Build history of the part. All positions in model axes, mm. Face numbers are marked on the shaded views. A direction names the side the tool comes from. Give positions to 0.01 mm unless a question says otherwise; leave off trailing zeros. Loops run counter-clockwise (first coordinate to the right, second up) from the corner with the lowest first, then second, coordinate; pieces in that order, holes last. Notation, with made-up numbers: (59, -37) -> (92, -37) arc R11 ccw to (92, -32) -> close; hole circle Ø2 at (-36, 2.25). An arc over 180 degrees is marked (long way). Answer in a Markdown table with one row per item. Add a question column.
from build123d import *

# Parameters (mm, degrees)
SKETCH_1_R      = 20
SKETCH_1_R_2    = 10
EXTRUDE_1_DEPTH = 10
EXTRUDE_START   = 50
EXTRUDE_2_DEPTH = 50
SKETCH_4_R      = 5
EXTRUDE_3_DEPTH = 10


with BuildPart() as part:
    # 草图1 → 凸台-拉伸1 (new body)
    with BuildSketch(Plane.XY):
        with BuildLine():
            Line((0, 80), (-500, 80))
            ThreePointArc((-500, 80), (-580, 0), (-500, -80))
            Line((-500, -80), (0, -80))
            ThreePointArc((0, -80), (80, 0), (0, 80))
        make_face()
        Circle(SKETCH_1_R, mode=Mode.SUBTRACT)
        with Locations((-500, 0)):
            Circle(SKETCH_1_R_2, mode=Mode.SUBTRACT)
    extrude(amount=EXTRUDE_1_DEPTH)

    # 草图2 → 凸台-拉伸2 (add)
    with BuildSketch(Plane(origin=(0, 0, 0), x_dir=(-1, 0, 0), z_dir=(0, 0, -1)).offset(EXTRUDE_START)):
        with BuildLine():
            Line((0, -80), (500, -80))
            ThreePointArc((500, -80), (580, 0), (500, 80))
            Line((500, 80), (0, 80))
            ThreePointArc((0, 80), (-80, 0), (0, -80))
        make_face()
        with BuildLine():
            Line((0, -70), (500, -70))
            ThreePointArc((500, -70), (570, 0), (500, 70))
            Line((500, 70), (0, 70))
            ThreePointArc((0, 70), (-70, 0), (0, -70))
        make_face(mode=Mode.SUBTRACT)
    extrude(amount=-EXTRUDE_2_DEPTH)

    # 草图4 → 凸台-拉伸3 (add)
    with BuildSketch(Plane(origin=(0, 0, -50), x_dir=(-1, 0, 0), z_dir=(0, 0, -1))):
        with BuildLine():
            Line((0, 110), (0, 80))
            Line((0, 80), (30, 80))
            Line((30, 80), (30, 110))
            ThreePointArc((30, 110), (15, 125), (0, 110))
        make_face()
        with Locations((15, 110)):
            Circle(SKETCH_4_R, mode=Mode.SUBTRACT)
    extrude(amount=-EXTRUDE_3_DEPTH)


solid = part.part
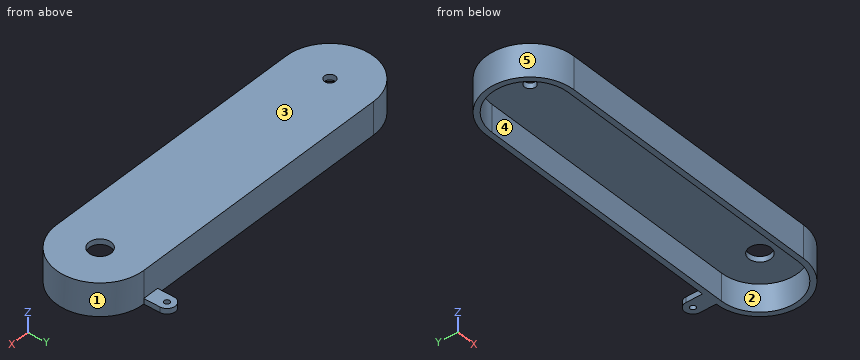
(1) Saw through at A-A, the plane y = 0. List the corners of the cut face in (x, z).
(2) Saw through at C-C, the plane x = -484. List the corners of the cut face in (y, z).
(3) Saw through at B-B, the plane z = -19.5. List the corners of the cut face in (x, y).
(4) Flat gauge pins, fed straight in: pin 1 Ø9 at (x, y) = (-18.5, 108) entering from +Z; pin 2 Ø8 at (y, z) = (20, -11.5) entering from +X; pin 3 Ø12 at (x, y) = (-500, 0) entering from +Z; pin 4 Ø5 at (x, z) = (-446.5, -40.5) entering from +Y. Where does each tip first touch, or does it go through?
(5) 3-axis set-ups, long thin cutter, end or side, ignore diameter. For the marked faces 4 and 5: which of +Z, -Z, +X, -X, +Y, -Y reach the whole face in a straight line?
(6) Saw through at D-D, the plane y = 42. List the corners of the cut face in (x, z), then the cut area to 3 significant figures.
(7) Wall check: line 1 along Y through (x, z) = (-15, -46); line 2 along Y through (x, z) = (-323, -32.5); line 3 along Y through (x, z) = (-500, 7). Give the ranges that are in metal, low to high. Write a range as from..to.
(8) Two-plate mould, pull along Y, no slides. Class the marked faces 1, 2 and 3: released by +Y, released by -Y, zero draft, split by the parting line, or undercut.
Worked answers:
| question | item | result |
|---|---|---|
| 1 | outline | (-580, -50) -> (-570, -50) -> (-570, 0) -> (-510, 0) -> (-510, 10) -> (-580, 10) -> close; (-490, 0) -> (-20, 0) -> (-20, 10) -> (-490, 10) -> close; (20, 0) -> (70, 0) -> (70, -50) -> (80, -50) -> (80, 10) -> (20, 10) -> close |
| 2 | outline | (-80, -50) -> (-70, -50) -> (-70, 0) -> (70, 0) -> (70, -50) -> (80, -50) -> (80, 10) -> (-80, 10) -> close |
| 3 | outline | (-500, -80) -> (0, -80) arc R80 ccw to (0, 80) -> (-500, 80) arc R80 ccw to start; hole (-500, -70) -> (0, -70) arc R70 ccw to (0, 70) -> (-500, 70) arc R70 ccw to start |
| 4 | pin 1 | z = -40 |
| 4 | pin 2 | x = 78.38 |
| 4 | pin 3 | through |
| 4 | pin 4 | y = 80 |
| 5 | face 4 | -Z |
| 5 | face 5 | +Z, -Z, -X |
| 6 | outline | (-568.09, -50) -> (-556, -50) -> (-556, 0) -> (56, 0) -> (56, -50) -> (68.09, -50) -> (68.09, 10) -> (-568.09, 10) -> close |
| 6 | area | 7,570 mm^2 |
| 7 | line 1 | -80..-70, 70..105, 115..125 |
| 7 | line 2 | -80..-70, 70..80 |
| 7 | line 3 | -80..-10, 10..80 |
| 8 | face 1 | split by the parting line |
| 8 | face 2 | undercut |
| 8 | face 3 | zero draft |
